CAD build for the part. Positions are in the model's coordinates, mm. Give positions to 0.01 mm unless a question says otherwise; leave off trailing zeros. Write each loop counter-clockwise with the first axis right and the second up, starting at its lowest first coordinate (ties: lowest second). Pieces come first, ordered by that corner, then holes. Notation, with made-up numbers: (22, 26) - (66, 26) arc R6 ccw to (66, 31) - close; hole circle Ø11 at (86, 29). An arc over 180 degrees is marked (long way). Answer as a JSON object with one key per item and string values.
from build123d import *

# Parameters (mm, degrees)
SKETCH1_R               = 500
BOSS_EXTRUDE1_DEPTH     = 50
CUT_EXTRUDE1_DEPTH      = 709.872343938
CUT_EXTRUDE1_DEPTH_BACK = 709.872343938
SKETCH2_W               = 450
SKETCH2_H               = 500


with BuildPart() as part:
    # Sketch1 → Boss-Extrude1 (new body)
    with BuildSketch(Plane(origin=(0, 0, 0), x_dir=(1, 0, 0), z_dir=(0, 1, 0))):
        with Locations(Location((0, 0, 0), (0, 0, 270))):
            Circle(SKETCH1_R)
    extrude(amount=BOSS_EXTRUDE1_DEPTH)

    # Sketch2 → Cut-Extrude1 (cut, two sides: drawn at the far end of the back side and taken through both)
    with BuildSketch(Plane(origin=(0, 50, 0), x_dir=(1, 0, 0), z_dir=(0, 1, 0)).offset(-CUT_EXTRUDE1_DEPTH_BACK)):
        Rectangle(SKETCH2_W, SKETCH2_H)
    extrude(amount=CUT_EXTRUDE1_DEPTH + CUT_EXTRUDE1_DEPTH_BACK, mode=Mode.SUBTRACT)


solid = part.part
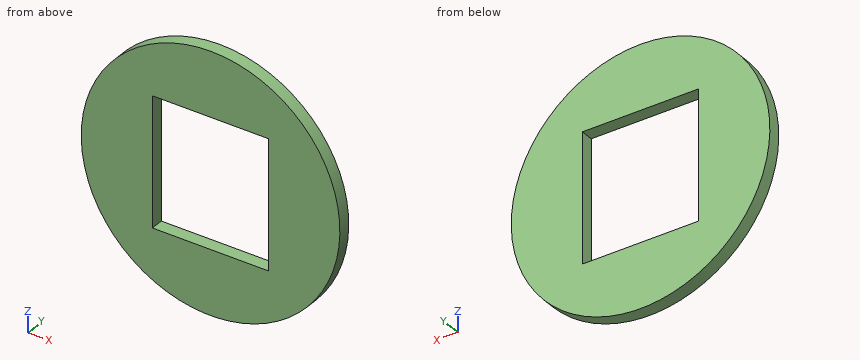
(1) Probe L1, parallel to Z at x = 223.5, y = 11.5; L2, parallel to Z at x = -53, y = 23; L3, parallel to X at y = 3, z = 176.5. List the from-to ranges inside material, lowest first. Write a range as [from, to].
Answer key:
{"L1": "z = [-447.27, -250], [250, 447.27]", "L2": "z = [-497.18, -250], [250, 497.18]", "L3": "x = [-467.81, -225], [225, 467.81]"}
(2) Saw through at C-C, the plane y = 7.5. Give the cut face in (x, z).
Answer key:
{"outline": "circle Ø1000 at (0, 0); hole (-225, -250) - (225, -250) - (225, 250) - (-225, 250) - close"}
(3) Saw through at D-D, the plane z = 411. Give the cut face in (x, y).
Answer key:
{"outline": "(-284.74, 0) - (284.74, 0) - (284.74, 50) - (-284.74, 50) - close"}
(4) Saw through at B-B, the plane z = 0. Give the cut face in (x, y), and give its area (3 significant figures).
Answer key:
{"outline": "(-500, 0) - (-225, 0) - (-225, 50) - (-500, 50) - close; (225, 0) - (500, 0) - (500, 50) - (225, 50) - close", "area": "27,500 mm²"}
(5) Saw through at A-A, the plane x = 0. Give the cut face in (y, z), and give its area (3 significant figures).
Answer key:
{"outline": "(0, -500) - (50, -500) - (50, -250) - (0, -250) - close; (0, 250) - (50, 250) - (50, 500) - (0, 500) - close", "area": "25,000 mm²"}
(6) Flat gauge pins, fed straight in: P1, Ø4, axis at y = 39, z = 378.5, coming from the -X side; P2, Ø6, axis at y = 19, z = -241.5, coming from the +X side; P3, Ø1, axis at x = -111, y = 29, coming from the -Z side. Where does each tip first touch, or does it go through?
Answer key:
{"P1": "stops at x = -329.01", "P2": "stops at x = 439.45", "P3": "stops at z = -487.64"}
